Geometry: final body of the model. Coordinates: model frame, mm. A direction names the side the tool comes from. Round coordinates to 2 decimals unless told otherwise and drop trailing zeros. Loops run counter-clockwise (first coordinate to the right, second up) from the corner with the lowest first, then second, coordinate; pieces in that order, holes last. Notation, with made-up numbers: M 64,-35 L 76,-35 A36 cw 76,0 Z; hole C 31,22.5 d3. An arc over 180 degrees is marked long. Return JSON: item names as keys, results as strings.
from build123d import *

# Parameters (mm, degrees)
BOSS_EXTRUDE1_DEPTH = 65
SKETCH3_R           = 50
SKETCH3_R_2         = 37.5
BOSS_EXTRUDE2_DEPTH = 65
SKETCH4_R           = 37.5
CUT_EXTRUDE2_DEPTH  = 130


with BuildPart() as part:
    # Sketch1 → Boss-Extrude1 (new body)
    with BuildSketch(Plane.XY):
        Polygon((77.5, 44.744645862), (0, 89.489291724), (-77.5, 44.744645862), (-77.5, -44.744645862), (0, -89.489291724), (77.5, -44.744645862), align=None)
    extrude(amount=BOSS_EXTRUDE1_DEPTH)

    # Sketch2 → Cut-Revolve1 (revolve, cut)
    with BuildSketch(Plane(origin=(0, 0, 0), x_dir=(0, 0, -1), z_dir=(1, 0, 0)), mode=Mode.PRIVATE) as cut_revolve1_sk:
        with BuildLine():
            Line((0, 59.489291724), (0, 89.489291724))
            Line((0, 89.489291724), (-30, 89.489291724))
            ThreePointArc((-30, 89.489291724), (-8.786796564, 80.70249516), (0, 59.489291724))
        make_face()
    revolve(cut_revolve1_sk.sketch.rotate(Axis((0, 0, 90.10395437), (0, 0, -1)), 90), axis=Axis((0, 0, 90.10395437), (0, 0, -1)), mode=Mode.SUBTRACT)

    # Sketch3 → Boss-Extrude2 (add)
    with BuildSketch(Plane(origin=(0, 0, 0), x_dir=(-1, 0, 0), z_dir=(0, 0, -1))):
        with Locations(Location((0, 0, 0), (0, 0, 180))):
            Circle(SKETCH3_R)
        Circle(SKETCH3_R_2, mode=Mode.SUBTRACT)
    extrude(amount=BOSS_EXTRUDE2_DEPTH)

    # Sketch4 → Cut-Extrude2 (cut)
    with BuildSketch(Plane.XY.offset(65)):
        Circle(SKETCH4_R)
    extrude(amount=-CUT_EXTRUDE2_DEPTH, mode=Mode.SUBTRACT)


solid = part.part
Q1. Section query B-B (z = 41). Output: boundary loops of the cut face in (x, y), plus the area to 3 significant figures.
Determined:
{"outline": "M -77.5,-44.74 L 0,-89.49 L 77.5,-44.74 L 77.5,44.74 L 0,89.49 L -77.5,44.74 Z; hole C 0,0 d75", "area": "16,400 mm^2"}
Q2. Pull-direction query (X, two-part tool) for faces 1 (the cylindrical face through (-4.88, 37.18, 0.91)), 2 (the flat face through (-38.21, 67.43, 35.09)), 3 (the flat face through (-1, -39, 65)); classes: pulls with the +X half, pulls with the -X half, needs draft (parallel to the pull), parting line crosses it, or undercut.
Determined:
{"face 1": "undercut", "face 2": "pulls with the -X half", "face 3": "needs draft"}
Q3. Pin query (flat end, axial travel): pin 1 (1 mm diameter, centred on x = 41, z = -23, fed in from -Y); pin 2 (1 mm diameter, centred on x = -19, z = 30, fed in from -Y); pin 3 (3 mm diameter, centred on x = -24, z = -46, fed in from +Y). Return the tip coordinate at first contact, or that it passes through.
Determined:
{"pin 1": "stops at y = -29.32", "pin 2": "stops at y = -78.81", "pin 3": "stops at y = 44.65"}
Q4. Reachability of faces 4 (the flat face through (38.21, -67.43, 35.09)), 5 (the cylindrical face through (47.69, -15.02, -32.04)) from +Z, -Z, +X, -X, +Y, -Y: full face, straight path, thin tool, end or side. Return the list, or none.
Determined:
{"face 4": "+Z, -Z, +X, -Y", "face 5": "-Z"}
Q5. Material intervals for L1, parallel to Y at x = 0, z = -34; L2, parallel to X at y = 0, z = 30; L3, parallel to Z at x = -46.5, y = -21, sorted ascending.
Determined:
{"L1": "y = -50 to -37.5, 37.5 to 50", "L2": "x = -77.5 to -37.5, 37.5 to 77.5", "L3": "z = 0 to 65"}
Q6. Section query C-C (z = -33.5). Output: boundary loops of the cut face in (x, y).
Determined:
{"outline": "C 0,0 d100; hole C 0,0 d75"}
Q7. Section query A-A (y = 0). Output: boundary loops of the cut face in (x, z).
Determined:
{"outline": "M -77.5,6.01 A30 ccw -59.49,0 L -50,0 L -50,-65 L -37.5,-65 L -37.5,65 L -77.5,65 Z; M 37.5,-65 L 50,-65 L 50,0 L 59.49,0 A30 ccw 77.5,6.01 L 77.5,65 L 37.5,65 Z"}
